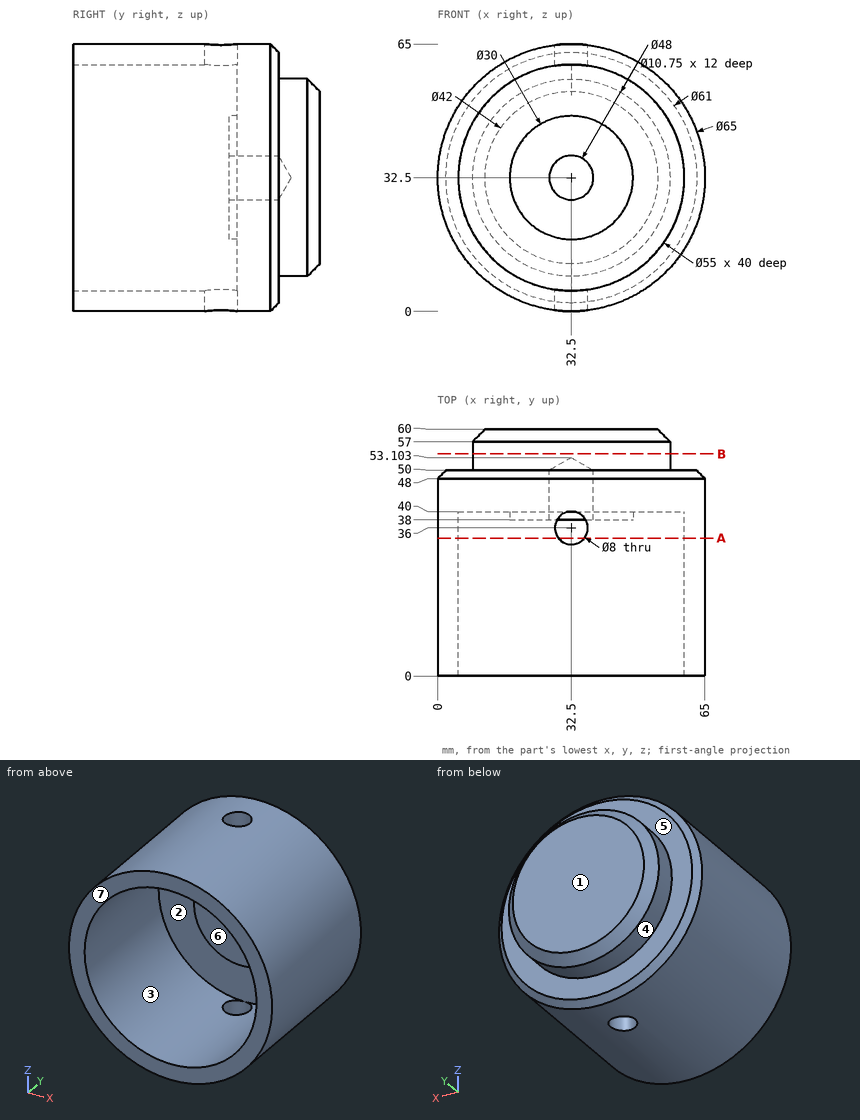
The drawing under review shows one solid part. Ordinate dimensions are in mm from its lowest x, y, z. A direction names the side the tool comes from. Give positions to 0.01 mm unless a question says otherwise; leave off trailing zeros. Loops run counter-clockwise (first coordinate to the right, second up) from the corner with the lowest first, then second, coordinate; pieces in that order, holes last. Notation, with made-up numbers: M 85.5,-4 L 126.5,-4 A15 ccw 126.5,7 Z; hole C 68,29.25 d6. An arc over 180 degrees is marked long. One line per item, written item: value. Start each with the question number.
Q1. Add section A-A (y = 33.5). Give the boundary of the cut face in (x, z), and give its area (3 significant figures).
Q2. Machinability: for the marked faces 5, 6 and 7, which of the approach directions +Z, -Z, +X, -X, +Y, -Y give a long, thin tool a straight path to every point of the face, cutting with its end or side? Answer none if there is none.
Q3. Clearance check with flat-ended pins moving along their axes: pin 1 Ø4 at (y, z) = (26, 36) entering from -X; pin 2 Ø15 at (x, z) = (29.5, 31) entering from -Y; pin 3 Ø12 at (x, y) = (9, 33.5) entering from +Z. State where each tip first meets the part, or that it passes through.
Q4. For L1, parallel to Z at x = 32, y = 23 (1 decimal); L2, parallel to Y at x = 28, z = 5.5; L3, parallel to Y at x = 39, z = 39, list the stretches that pass through material, from the lowest coordinate up.
Q5. Add section B-B (y = 54). Give the boundary of the cut face in (x, z).
Q6. Draft analysis for pull direction X (two halves, no side actions). For the marked faces 1, 2, 3 and 4, state which applies: released by +X, released by -X, zero draft, split by the parting line, or undercut.
Reply:
1. outline: M 29.38,0.15 L 29.38,5.18 A27.5 cw 29.38,59.82 L 29.38,64.85 A32.5 ccw Z; M 35.62,0.15 A32.5 ccw 35.62,64.85 L 35.62,59.82 A27.5 cw 35.62,5.18 Z
1. area: 880 mm²
2. face 5: +Y
2. face 6: -Y
2. face 7: +Z, -Z, +X, -X, -Y
3. pin 1: x = 0.03
3. pin 2: y = 38
3. pin 3: z = 59.89
4. L1: 0 to 5, 60 to 65
4. L2: 40 to 50
4. L3: 38 to 60
5. outline: C 32.5,32.5 d48
6. face 1: zero draft
6. face 2: undercut
6. face 3: undercut
6. face 4: split by the parting line
